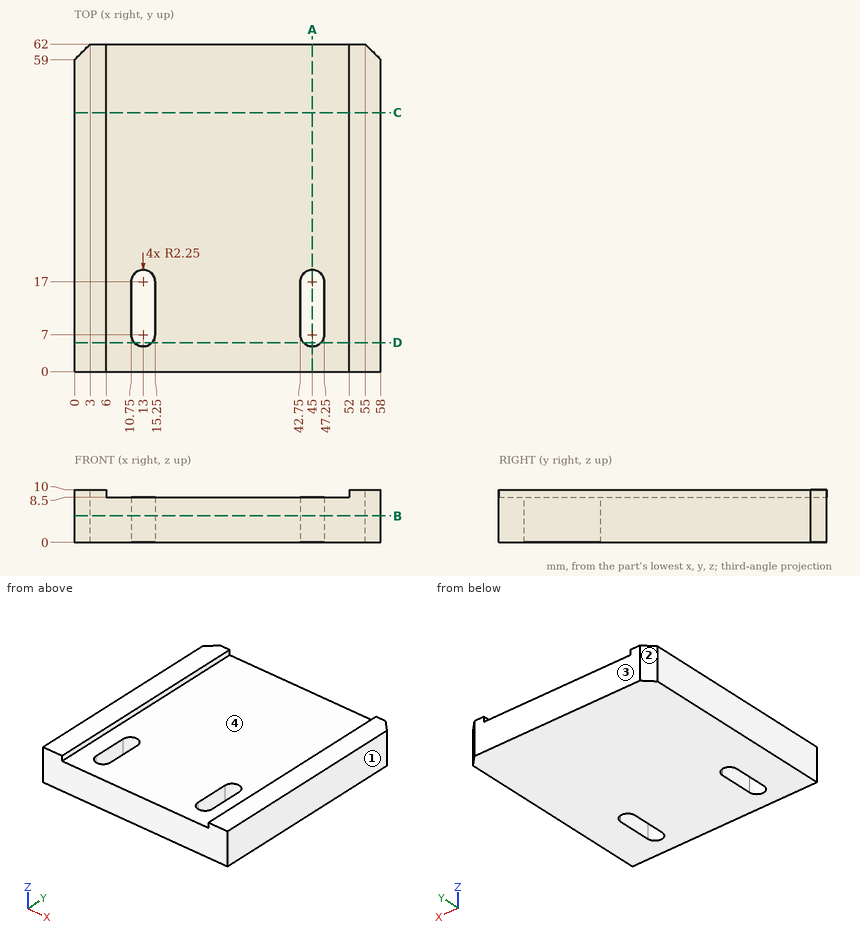
Check sheet for the drawn part. Datum: minimum x, y, z corner. Units: mm. Coordinates: 2 decimals unless noted, no trailing zeros. Loops run counter-clockwise (first coordinate to the right, second up) from the corner with the lowest first, then second, coordinate; pieces in that order, holes last. Notation, with made-up numbers: (-2.75, 71) -> (41.25, 71) arc R18 ccw to (41.25, 99) -> close; hole circle Ø6 at (86, 20.25). An arc over 180 degrees is marked (long way). Answer as a JSON object with one key per item and string values. Group by question number.
Item 1: Scan lines: probe 1 along X at (y, z) = (15, 7); probe 2 along X at (y, z) = (38.5, 9.25); probe 3 along Z at (x, y) = (51, 30). Record each from-to range of solid material in increasing order.
Item 2: Sectioned sample at D-D on y = 5.5. Record the boundary of the cut face in (x, z).
Item 3: Mould release check, pull along X, two halves, no side actions. Record for the marked faces 1, 2, 3 and 4: +X half, -X half, draft (parallel to the pull), parting line (faces both ways), or undercut.
Item 4: Sectioned sample at B-B on z = 5. Record the boundary of the cut face in (x, y), plus the area to 3 significant figures.
Item 5: Sectioned sample at A-A on x = 45. Record the boundary of the cut face in (y, z).
Item 6: Sectioned sample at C-C on y = 49. Record the boundary of the cut face in (x, z).
Item 7: Depth check by flat-ended pin: pin 1 (1 mm diameter, centred on x = 11.5, z = 5.5, fed in from -Y). Enter the tip coordinate at first touch or a pass-through.
Evaluation:
{
 "1": {"probe 1": "x = 0 to 10.75, 15.25 to 42.75, 47.25 to 58", "probe 2": "x = 0 to 6, 52 to 58", "probe 3": "z = 0 to 8.5"},
 "2": {"outline": "(0, 0) -> (11.32, 0) -> (11.32, 8.5) -> (6, 8.5) -> (6, 10) -> (0, 10) -> close; (14.68, 0) -> (43.32, 0) -> (43.32, 8.5) -> (14.68, 8.5) -> close; (46.68, 0) -> (58, 0) -> (58, 10) -> (52, 10) -> (52, 8.5) -> (46.68, 8.5) -> close"},
 "3": {"face 1": "+X half", "face 2": "-X half", "face 3": "draft", "face 4": "undercut"},
 "4": {"outline": "(0, 0) -> (58, 0) -> (58, 59) -> (55, 62) -> (3, 62) -> (0, 59) -> close; hole (10.75, 7) arc R2.25 ccw to (15.25, 7) -> (15.25, 17) arc R2.25 ccw to (10.75, 17) -> close; hole (42.75, 7) arc R2.25 ccw to (47.25, 7) -> (47.25, 17) arc R2.25 ccw to (42.75, 17) -> close", "area": "3,470 mm²"},
 "5": {"outline": "(0, 0) -> (4.75, 0) -> (4.75, 8.5) -> (0, 8.5) -> close; (19.25, 0) -> (62, 0) -> (62, 8.5) -> (19.25, 8.5) -> close"},
 "6": {"outline": "(0, 0) -> (58, 0) -> (58, 10) -> (52, 10) -> (52, 8.5) -> (6, 8.5) -> (6, 10) -> (0, 10) -> close"},
 "7": {"pin 1": "stops at y = 0"}
}
